Check sheet for the modelled part. Datum: model origin and axes. Units: mm. A direction names the side the tool comes from. Round coordinates to 2 decimals unless told otherwise and drop trailing zeros. Write each loop counter-clockwise with the first axis right and the second up, starting at its lowest first coordinate (ties: lowest second). Pieces come first, ordered by that corner, then holes. Notation, with made-up numbers: (-38.5, 16) - (9.5, 16) arc R24 ccw to (9.5, 52) - close; hole circle Ø1 at (-11, 76.5). An arc over 180 degrees is marked (long way). Use one line per item in the form item = value. Start each with the question number.
1) Section check D-D (x = -14). Record the boundary of the cut face in (y, z), then the cut area to 3 significant figures.
2) Draft check along Y on faces 3 (the face through (35, 0, 1)), 4 (the face through (24.5, 0.1, 1)), 5 (the face through (34, -36, 1)). Enter one of: +Y half, -Y half, draft (parallel to the pull), parting line (faces both ways), or undercut.
3) Section check C-C (y = -22). Record the boundary of the cut face in (x, z).
4) Scan lines: probe 1 along Y at (x, z) = (-27, 1.1); probe 2 along X at (y, z) = (3.5, 0.9); probe 3 along Y at (x, z) = (-15, 1.7). Record each from-to range of solid material in increasing order.
5) Gauge pin test, flat end, axial feed: P1, Ø4.5, axis at x = -27, y = 0, coming from the +Z side. Record the tip position at first contact, or that the pin passes through.
6) Section check A-A (x = 27). Record the boundary of the cut face in (y, z), then the cut area to 3 significant figures.
7) Set-up check for faces 1 (the face through (34, 36, 1)), 2 (the face through (22, 0, 1)): record each of +Z, -Z, +X, -X, +Y, -Y from which the full face is reachable in a straight line by a thin tool's end or side.
8) Section check B-B (y = -30). Record the boundary of the cut face in (x, z), then the cut area to 3 significant figures.
from build123d import *

# Parameters (mm, degrees)
SKETCH1_W           = 70
SKETCH1_H           = 74
SKETCH1_R           = 2.5
BOSS_EXTRUDE1_DEPTH = 2
CHAMFER1_SIZE       = 2


with BuildPart() as part:
    # Sketch1 → Boss-Extrude1 (new body)
    with BuildSketch(Plane.XY):
        Rectangle(SKETCH1_W, SKETCH1_H)
        with Locations((-27, 30)):
            Circle(SKETCH1_R, mode=Mode.SUBTRACT)
        with Locations((-27, 0)):
            Circle(SKETCH1_R, mode=Mode.SUBTRACT)
        with Locations((-27, -30)):
            Circle(SKETCH1_R, mode=Mode.SUBTRACT)
        with Locations((27, -30)):
            Circle(SKETCH1_R, mode=Mode.SUBTRACT)
        with Locations((27, 0)):
            Circle(SKETCH1_R, mode=Mode.SUBTRACT)
        with Locations((27, 30)):
            Circle(SKETCH1_R, mode=Mode.SUBTRACT)
        with BuildLine():
            Line((-19, -34.5), (19, -34.5))
            ThreePointArc((19, -34.5), (21.121320344, -33.621320344), (22, -31.5))
            Line((22, -31.5), (22, 31.5))
            ThreePointArc((22, 31.5), (21.121320344, 33.621320344), (19, 34.5))
            Line((19, 34.5), (-19, 34.5))
            ThreePointArc((-19, 34.5), (-21.121320344, 33.621320344), (-22, 31.5))
            Line((-22, 31.5), (-22, -31.5))
            ThreePointArc((-22, -31.5), (-21.121320344, -33.621320344), (-19, -34.5))
        make_face(mode=Mode.SUBTRACT)
    extrude(amount=BOSS_EXTRUDE1_DEPTH)

    # Chamfer1
    chamfer1_edges = [part.edges().sort_by_distance(p)[0] for p in [
        (35, -37, 1),
        (-35, -37, 1),
        (-35, 37, 1),
        (35, 37, 1),
    ]]
    chamfer(chamfer1_edges, length=CHAMFER1_SIZE)


solid = part.part
Results are:
q1.outline = (-37, 0) - (-34.5, 0) - (-34.5, 2) - (-37, 2) - close; (34.5, 0) - (37, 0) - (37, 2) - (34.5, 2) - close
q1.area = 10.0 mm²
q2.face_3 = draft
q2.face_4 = undercut
q2.face_5 = -Y half
q3.outline = (-35, 0) - (-22, 0) - (-22, 2) - (-35, 2) - close; (22, 0) - (35, 0) - (35, 2) - (22, 2) - close
q4.probe_1 = -37 to -32.5, -27.5 to -2.5, 2.5 to 27.5, 32.5 to 37
q4.probe_2 = -35 to -22, 22 to 35
q4.probe_3 = -37 to -34.5, 34.5 to 37
q5.P1 = through
q6.outline = (-37, 0) - (-32.5, 0) - (-32.5, 2) - (-37, 2) - close; (-27.5, 0) - (-2.5, 0) - (-2.5, 2) - (-27.5, 2) - close; (2.5, 0) - (27.5, 0) - (27.5, 2) - (2.5, 2) - close; (32.5, 0) - (37, 0) - (37, 2) - (32.5, 2) - close
q6.area = 118 mm²
q7.face_1 = +Z, -Z, +X, +Y
q7.face_2 = +Z, -Z
q8.outline = (-35, 0) - (-29.5, 0) - (-29.5, 2) - (-35, 2) - close; (-24.5, 0) - (-22, 0) - (-22, 2) - (-24.5, 2) - close; (22, 0) - (24.5, 0) - (24.5, 2) - (22, 2) - close; (29.5, 0) - (35, 0) - (35, 2) - (29.5, 2) - close
q8.area = 32.0 mm²
